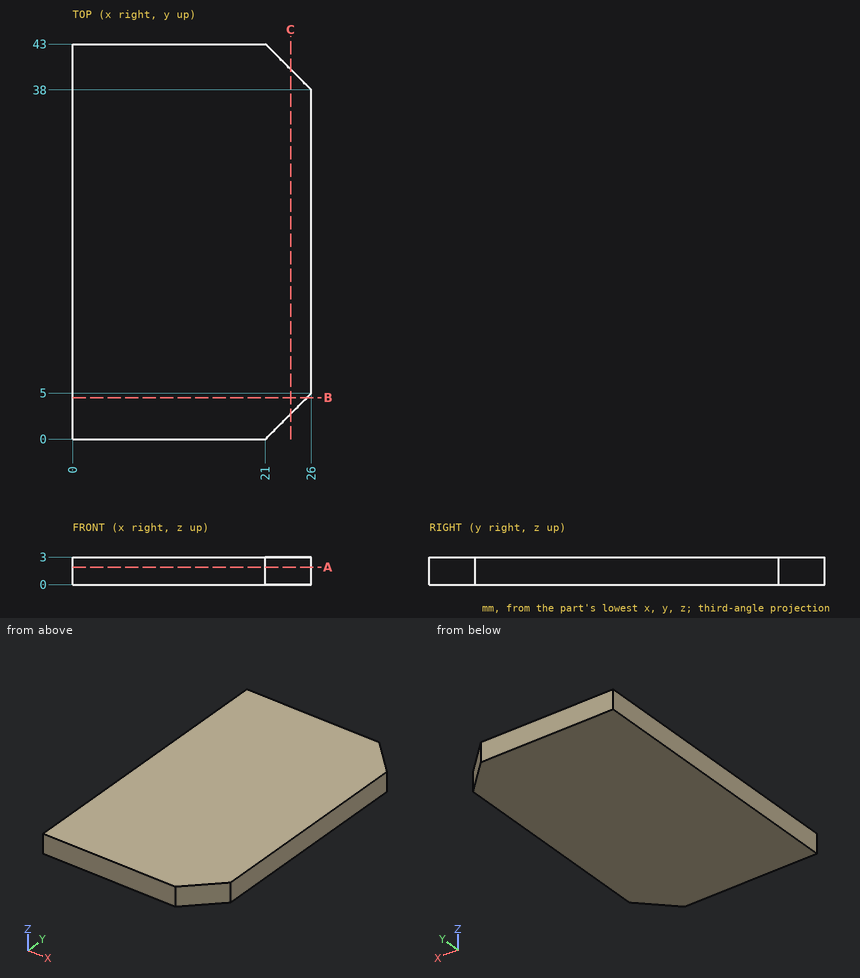
Part print with two shaded views. Sizes in mm from the minimum x, y, z corner. Coordinates: 2 decimals unless noted, no trailing zeros. Loops run counter-clockwise (first coordinate to the right, second up) from the corner with the lowest first, then second, coordinate; pieces in that order, holes last. Notation, with made-up numbers: (-6.5, -21) - (12.5, -21) arc R25 ccw to (12.5, -6) - close; hole circle Ø4 at (83, -23). An arc over 180 degrees is marked (long way). Write each question's results on one line, items separated by ' | '. Start each with the question number.
Q1. Slice it at C-C on x = 23.75. Give the cut face in (y, z), and give its area (4 significant figures).
Q2. Slice it at B-B on y = 4.5. Give the cut face in (x, z).
Q3. Slice it at A-A on z = 1.9. Give the cut face in (x, y), and give its area (3 significant figures).
Q4. Probe line 1 along X through (y, z) = (39.5, 1.4); line 2 along Y through (x, z) = (23.5, 1.85); line 3 along Y through (x, z) = (23, 0.1). List the from-to ranges inside material, lowest first.
Answer:
1) outline: (2.75, 0) - (40.25, 0) - (40.25, 3) - (2.75, 3) - close | area: 112.5 mm2
2) outline: (0, 0) - (25.5, 0) - (25.5, 3) - (0, 3) - close
3) outline: (0, 0) - (21, 0) - (26, 5) - (26, 38) - (21, 43) - (0, 43) - close | area: 1,090 mm2
4) line 1: x = 0 to 24.5 | line 2: y = 2.5 to 40.5 | line 3: y = 2 to 41
